```python
from build123d import *

# Parameters (mm, degrees)
SKETCH_1_W      = 247
SKETCH_1_H      = 19
EXTRUDE_1_DEPTH = 2.5
CHAMFER_1_SIZE  = 10


with BuildPart() as part:
    # 草图1 → 凸台-拉伸1 (new, symmetric)
    with BuildSketch(Plane(origin=(0, 0, 0), x_dir=(0, 0, -1), z_dir=(1, 0, 0))):
        Rectangle(SKETCH_1_W, SKETCH_1_H)
    extrude(amount=EXTRUDE_1_DEPTH, both=True)

    # 倒角1
    chamfer_1_edges = [part.edges().sort_by_distance(p)[0] for p in [
        (0, -9.5, -123.5),
        (0, -9.5, 123.5),
    ]]
    chamfer(chamfer_1_edges, length=CHAMFER_1_SIZE)


solid = part.part
```
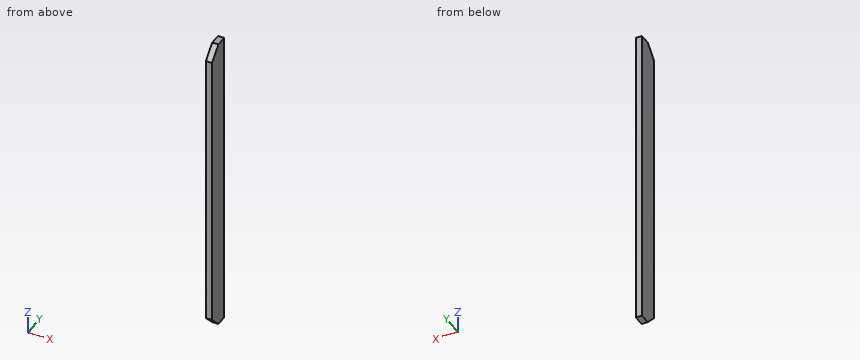
Here's how the part is built. I have some questions about the finished solid (model axes, mm). Coordinates: 2 decimals unless noted, no trailing zeros. Order: outer loops, then holes, each group sorted by start corner. A loop starts at its lowest first (then second) coordinate and runs counter-clockwise, first axis right, second up. Notation, with made-up numbers: M 49,-23 L 92,-23 A23 ccw 92,-6 Z; hole C 18.25,-18.75 d6. An arc over 180 degrees is marked long. Answer as a JSON object with one key per item and string values. Group by question number.
(1) Suppose I cut it at A-A, the plane x = -0.9. Please give me the cut outline in (y, z), then the cut area to 3 significant figures.
(2) Suppose I cut it at B-B, the plane y = -5.25. Please give me the cut outline in (x, z).
(3) I need wall thicknesses on probe 1 along Z at (x, y) = (1.1, -2.75); probe 2 along Z at (x, y) = (0.95, -3). Which ranges of each line are inside material? Lowest first, please.
Values found:
{
 "1": {"outline": "M -9.5,-113.5 L 0.5,-123.5 L 9.5,-123.5 L 9.5,123.5 L 0.5,123.5 L -9.5,113.5 Z", "area": "4,590 mm^2"},
 "2": {"outline": "M -2.5,-117.75 L 2.5,-117.75 L 2.5,117.75 L -2.5,117.75 Z"},
 "3": {"probe 1": "z = -120.25 to 120.25", "probe 2": "z = -120 to 120"}
}
